Part model, mm, in its own coordinate system. A direction names the side the tool comes from. Give positions to 0.01 mm unless a question says otherwise; leave off trailing zeros. Loops run counter-clockwise (first coordinate to the right, second up) from the corner with the lowest first, then second, coordinate; pieces in that order, holes last. Notation, with made-up numbers: (61, -22.75) -> (101, -22.75) arc R27 cw to (101, 8.25) -> close; hole circle Ø9 at (78, 62). An arc over 180 degrees is marked (long way). Write item = value, one per line.
from build123d import *

# Parameters (mm, degrees)
EXTRUDE_1_DEPTH          = 15
SKETCH_2_W               = 1
SKETCH_2_H               = 5
CUT_EXTRUDE_1_DEPTH      = 10.8
SKETCH_3_R               = 1.45
CUT_EXTRUDE_2_DEPTH      = 1
EXTRUDE_2_DEPTH          = 22
CUT_EXTRUDE_3_DEPTH      = 1.4
CUT_EXTRUDE_3_DEPTH_BACK = 1.4
SKETCH_5_W               = 0.5
SKETCH_5_H               = 5
SKETCH_6_R               = 1.25
SKETCH_6_R_2             = 1.05
CUT_EXTRUDE_4_DEPTH      = 0.1
CUT_EXTRUDE_5_DEPTH      = 0.1
CUT_EXTRUDE_6_DEPTH      = 0.1
SKETCH_9_R               = 1.35
EXTRUDE_3_DEPTH          = 10


with BuildPart() as part:
    # 草图1 → 凸台-拉伸1 (new body)
    with BuildSketch(Plane.XY):
        with BuildLine():
            Line((-2, -3.1), (1.6, -3.1))
            Line((1.6, -3.1), (1.946410162, -2.5))
            Line((1.946410162, -2.5), (3.9, -2.5))
            Line((3.9, -2.5), (3.9, 2.5))
            Line((3.9, 2.5), (1.946410162, 2.5))
            Line((1.946410162, 2.5), (1.6, 3.1))
            Line((1.6, 3.1), (-2, 3.1))
            Line((-2, 3.1), (-2, 2))
            Line((-2, 2), (0, 2))
            ThreePointArc((0, 2), (0.707106781, 1.870828693), (1.322875656, 1.5))
            Line((1.322875656, 1.5), (2.9, 1.5))
            Line((2.9, 1.5), (2.9, -1.5))
            Line((2.9, -1.5), (1.322875656, -1.5))
            ThreePointArc((1.322875656, -1.5), (0.707106781, -1.870828693), (0, -2))
            Line((0, -2), (-2, -2))
            Line((-2, -2), (-2, -3.1))
        make_face()
    extrude(amount=-EXTRUDE_1_DEPTH)

    # 草图2 → 切除-拉伸1 (cut)
    with BuildSketch(Plane.XY.offset(-4.2)):
        with Locations((3.4, 0)):
            Rectangle(SKETCH_2_W, SKETCH_2_H)
    extrude(amount=-CUT_EXTRUDE_1_DEPTH, mode=Mode.SUBTRACT)

    # 草图3 → 切除-拉伸2 (cut)
    with BuildSketch(Plane(origin=(3.9, 0, 0), x_dir=(0, 0, -1), z_dir=(1, 0, 0))):
        with Locations((2, 0)):
            Circle(SKETCH_3_R)
    extrude(amount=-CUT_EXTRUDE_2_DEPTH, mode=Mode.SUBTRACT)

    # 草图4 → 凸台-拉伸2 (add)
    with BuildSketch(Plane.XY):
        with BuildLine():
            Line((1.428285686, -1.4), (2.5, -1.4))
            Line((2.5, -1.4), (2.5, 1.4))
            Line((2.5, 1.4), (1.428285686, 1.4))
            ThreePointArc((1.428285686, 1.4), (-2, 0), (1.428285686, -1.4))
        make_face()
    extrude(amount=-EXTRUDE_2_DEPTH)

    # 草图5 → 切除-拉伸3 (cut, two sides: drawn at the far end of the back side and taken through both)
    with BuildSketch(Plane(origin=(0, 0, 0), x_dir=(1, 0, 0), z_dir=(0, 1, 0)).offset(-CUT_EXTRUDE_3_DEPTH_BACK)):
        with Locations((2.25, 2.5)):
            Rectangle(SKETCH_5_W, SKETCH_5_H)
    extrude(amount=CUT_EXTRUDE_3_DEPTH + CUT_EXTRUDE_3_DEPTH_BACK, mode=Mode.SUBTRACT)

    # 草图6 → 切除-拉伸4 (cut)
    with BuildSketch(Plane(origin=(2, 0, 0), x_dir=(0, 0, -1), z_dir=(1, 0, 0))):
        with Locations((2, 0)):
            Circle(SKETCH_6_R)
        with Locations((2, 0)):
            Circle(SKETCH_6_R_2, mode=Mode.SUBTRACT)
    extrude(amount=-CUT_EXTRUDE_4_DEPTH, mode=Mode.SUBTRACT)

    # 草图7 → 切除-拉伸5 (cut)
    with BuildSketch(Plane(origin=(2, 0, 0), x_dir=(0, 0, -1), z_dir=(1, 0, 0))):
        with BuildLine():
            Line((0.966284129, 0.609451802), (2.609451802, -1.033715871))
            ThreePointArc((2.609451802, -1.033715871), (2.848528137, -0.848528137), (3.033715871, -0.609451802))
            Line((3.033715871, -0.609451802), (1.390548198, 1.033715871))
            ThreePointArc((1.390548198, 1.033715871), (1.151471863, 0.848528137), (0.966284129, 0.609451802))
        make_face()
    extrude(amount=-CUT_EXTRUDE_5_DEPTH, mode=Mode.SUBTRACT)

    # 草图8 → 切除-拉伸6 (cut)
    with BuildSketch(Plane(origin=(2.5, 0, 0), x_dir=(0, 0, -1), z_dir=(1, 0, 0))):
        with BuildLine():
            Line((7.4, -0.8), (9.6, -0.8))
            ThreePointArc((9.6, -0.8), (9.882842712, -0.682842712), (10, -0.4))
            Line((10, -0.4), (10, 0.4))
            ThreePointArc((10, 0.4), (9.882842712, 0.682842712), (9.6, 0.8))
            Line((9.6, 0.8), (7.4, 0.8))
            ThreePointArc((7.4, 0.8), (7.117157288, 0.682842712), (7, 0.4))
            Line((7, 0.4), (7, -0.4))
            ThreePointArc((7, -0.4), (7.117157288, -0.682842712), (7.4, -0.8))
        make_face()
    extrude(amount=-CUT_EXTRUDE_6_DEPTH, mode=Mode.SUBTRACT)

    # 草图9 → 凸台-拉伸3 (add)
    with BuildSketch(Plane.XY.offset(-22)):
        Circle(SKETCH_9_R)
    extrude(amount=-EXTRUDE_3_DEPTH)


solid = part.part
1) Slice it at B-B, the plane y = 0. Count the separate pieces of the cut face and the enclosed holes in it, and give its area (3 significant figures).
Resolved:
separate_pieces = 3
enclosed_holes = 0
area = 124 mm²
2) Drop flat-ended pins along their axis: P1, Ø0.8, axis at y = -0.5, z = -2, coming from the +X side; P2, Ø1.3, axis at x = 0.5, y = 2, coming from the -Z side; P3, Ø1.5, axis at y = -2, z = -9, coming from the +X side; P4, Ø1, axis at x = 3.5, z = -6.5, coming from the -Y side. Give the stop position or say it passes through.
Resolved:
P1 = 2
P2 = -22
P3 = 2.9
P4 = through
3) Drill centre lines: line 1 along Z through (x, y) = (3.4, 1); line 2 along Y through (x, z) = (2.05, -2); line 3 along Y through (x, z) = (3.2, -2). Where is each one in solid material? Low to high. Write a range as [from, to].
Resolved:
line_1 = [-4.2, -3.05], [-0.95, 0]
line_2 = [-2.5, -1.5], [1.5, 2.5]
line_3 = [-2.5, -1.45], [1.45, 2.5]
4) Which spindle directions (+Z, -Z, +X, -X, +Y, -Y) get a long thin tool onto all of the face, cutting with end or side? Do faces 1 (the face through (2, -0.5, -1.5)), 2 (the face through (0.4, 2.5, -15)), 3 (the face through (2.4, 0, -8)). Say none if no direction does.
Resolved:
face_1 = +Z, +X
face_2 = -Z, +X, +Y
face_3 = +X
5) Slice it at A-A, the plane z = -8.5. List the corners of the cut face in (x, y), and give its area (3 significant figures).
Resolved:
outline = (-2, -3.1) -> (1.6, -3.1) -> (1.95, -2.5) -> (2.9, -2.5) -> (2.9, -1.5) -> (1.32, -1.5) arc R2 ccw to (1.43, -1.4) -> (2.5, -1.4) -> (2.5, -0.8) -> (2.4, -0.8) -> (2.4, 0.8) -> (2.5, 0.8) -> (2.5, 1.4) -> (1.43, 1.4) arc R2 ccw to (1.32, 1.5) -> (2.9, 1.5) -> (2.9, 2.5) -> (1.95, 2.5) -> (1.6, 3.1) -> (-2, 3.1) -> (-2, 2) -> (0, 2) arc R2 ccw to (0, -2) -> (-2, -2) -> close
area = 25.7 mm²
6) Slice it at D-D, the plane z = -4.5. List the corners of the cut face in (x, y).
Resolved:
outline = (-2, -3.1) -> (1.6, -3.1) -> (1.95, -2.5) -> (2.9, -2.5) -> (2.9, -1.5) -> (1.32, -1.5) arc R2 ccw to (1.43, -1.4) -> (2, -1.4) -> (2, 1.4) -> (1.43, 1.4) arc R2 ccw to (1.32, 1.5) -> (2.9, 1.5) -> (2.9, 2.5) -> (1.95, 2.5) -> (1.6, 3.1) -> (-2, 3.1) -> (-2, 2) -> (0, 2) arc R2 ccw to (0, -2) -> (-2, -2) -> close
7) Slice it at C-C, the plane x = 1. List the corners of the cut face in (y, z), and give its area (3 significant figures).
Resolved:
outline = (-3.1, -15) -> (-1.73, -15) -> (-1.73, -22) -> (-0.91, -22) -> (-0.91, -32) -> (0.91, -32) -> (0.91, -22) -> (1.73, -22) -> (1.73, -15) -> (3.1, -15) -> (3.1, 0) -> (-3.1, 0) -> close
area = 135 mm²
8) Pull direction Y, two halves, no side cores. Call faces 4 (the face through (-0.29, -1.32, -26.93)), 5 (the face through (3.41, 0.06, -0.55)), 6 (the face through (-2, -2.5, -7.4)): pulls with the +Y half, pulls with the -Y half, needs draft (parallel to the pull), parting line crosses it, or undercut.
Resolved:
face_4 = parting line crosses it
face_5 = undercut
face_6 = needs draft
